Model file for the job. Use its own axes, mm. Face numbers are marked on the shaded views. Round coordinates to 2 decimals unless told otherwise and drop trailing zeros. Use a Markdown table: item, result. Add a question column.
Item 1: Saw through at A-A on z = 0. Give the number of separate pieces and of enclosed holes in the cut face, then the cut area to 3 significant figures.
Item 2: Pin check, flat tips, straight feed: P1, Ø4, axis at x = 50, y = 7, coming from the +Z side; P2, Ø10, axis at y = -4.5, z = -1.5, coming from the -X side; P3, Ø5, axis at x = 11, y = -1.5, coming from the +Z side; P4, Ø8, axis at x = 26.5, z = -1, coming from the +Y side. Stop position of each tip, or through.
Item 3: Wall check: L1, parallel to X at y = 4.75, z = -0.25; L2, parallel to Y at x = 59, z = 0; L3, parallel to X at y = 9.5, z = -4. Give the ranges that are in metal, low to high. Write a range as from..to.
Item 4: Two-plate mould, pull along X, no slides. Class the marked faces 1, 2 and 3: +X half, -X half, draft (parallel to the pull), parting line (faces both ways), or undercut.
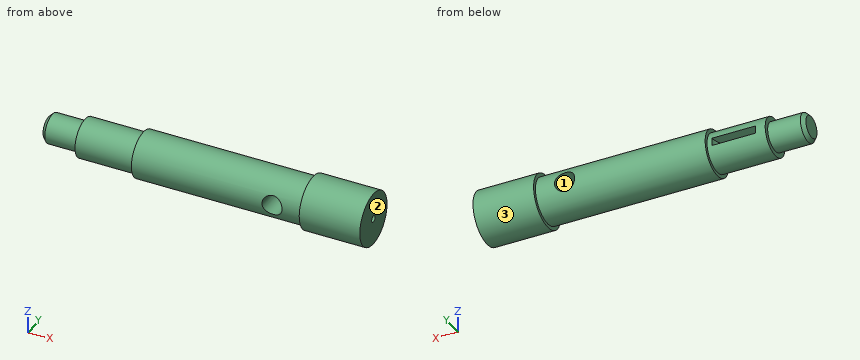
```python
from build123d import *

# Parameters (mm, degrees)
SKETCH2_R               = 1.4
CUT_EXTRUDE1_DEPTH      = 44
CUT_EXTRUDE2_DEPTH      = 84.095495831
CUT_EXTRUDE2_DEPTH_BACK = 84.095495831
SKETCH3_R               = 4.15
SKETCH5_W               = 9
SKETCH5_H               = 3.2
CHAMFER1_SIZE           = 1.5


with BuildPart() as part:
    # Sketch1 → Revolve1 (revolve)
    with BuildSketch(Plane(origin=(0, 0, 0), x_dir=(1, 0, 0), z_dir=(0, 1, 0)), mode=Mode.PRIVATE) as revolve1_sk:
        Polygon((-52.373647469, 0), (-52.373647469, 6), (-37.373647469, 6), (-37.373647469, 8), (-13.373647469, 8), (-13.373647469, 9.5), (56.626352531, 9.5), (56.626352531, 11), (81.626352531, 11), (81.626352531, 0), align=None)
    revolve(revolve1_sk.sketch.rotate(Axis((-52.373647469, 0, 0), (1, 0, 0)), 180), axis=Axis((-52.373647469, 0, 0), (1, 0, 0)))

    # Sketch2 → Cut-Extrude1 (cut)
    with BuildSketch(Plane(origin=(81.626352531, 0, 0), x_dir=(0, 0, -1), z_dir=(1, 0, 0))):
        Circle(SKETCH2_R)
    extrude(amount=-CUT_EXTRUDE1_DEPTH, mode=Mode.SUBTRACT)

    # Sketch3 → Cut-Extrude2 (cut, two sides: drawn at the far end of the back side and taken through both)
    with BuildSketch(Plane(origin=(0, 0, 0), x_dir=(1, 0, 0), z_dir=(0, 1, 0)).offset(-CUT_EXTRUDE2_DEPTH_BACK)):
        with Locations(Location((44.626352531, 0, 0), (0, 0, 270))):
            Circle(SKETCH3_R)
    extrude(amount=CUT_EXTRUDE2_DEPTH + CUT_EXTRUDE2_DEPTH_BACK, mode=Mode.SUBTRACT)

    # Sketch5 → Cut-Revolve3 (revolve, cut)
    with BuildSketch(Plane(origin=(0, 8, 0), x_dir=(-1, 0, 0), z_dir=(0, 1, 0))):
        with Locations((19.873647469, 0)):
            Rectangle(SKETCH5_W, SKETCH5_H)
    revolve(axis=Axis((-24.373647469, 8, 1.6), (0, 0, -1)), mode=Mode.SUBTRACT)

    # Chamfer1
    chamfer1_edges = [part.edges().sort_by_distance(p)[0] for p in [
        (-52.373647469, 0, -6),
    ]]
    chamfer(chamfer1_edges, length=CHAMFER1_SIZE)


solid = part.part
```
Entries:
| question | item | result |
|---|---|---|
| 1 | separate pieces | 3 |
| 1 | enclosed holes | 0 |
| 1 | area | 2,060 mm2 |
| 2 | P1 | z = 8.08 |
| 2 | P2 | x = -52.37 |
| 2 | P3 | z = 9.5 |
| 2 | P4 | y = 9.5 |
| 3 | L1 | -52.12..-32.77, -15.98..40.48, 48.77..81.63 |
| 3 | L2 | -11..-1.4, 1.4..11 |
| 3 | L3 | 56.63..81.63 |
| 4 | face 1 | undercut |
| 4 | face 2 | +X half |
| 4 | face 3 | draft |
